from build123d import *

# Parameters (mm, degrees)
M4_TAPPED_HOLE1_D     = 3.3
M4_TAPPED_HOLE1_DEPTH = 9.8
M4_TAPPED_HOLE1_TIP   = 0.991420021
CHAMFER1_SIZE         = 1


with BuildPart() as part:
    # Sketch1 → Revolve1 (revolve)
    with BuildSketch(Plane.XY, mode=Mode.PRIVATE) as revolve1_sk:
        Polygon((25, 0), (46.5, 0), (46.5, 4), (42.5, 4), (42.5, 14.5), (25, 14.5), align=None)
    revolve(revolve1_sk.sketch.rotate(Axis((0, 0, 0), (0, 1, 0)), 90), axis=Axis((0, 0, 0), (0, 1, 0)))

    # M4 Tapped Hole1
    with Locations(Plane(origin=(0, 0, 0), x_dir=(-1, 0, 0), z_dir=(0, -1, 0))):
        with Locations((0, -36.5), (-31.609927238, -18.25), (-31.609927238, 18.25), (0, 36.5), (31.609927238, 18.25), (31.609927238, -18.25)):
            Hole(M4_TAPPED_HOLE1_D / 2, depth=M4_TAPPED_HOLE1_DEPTH)
            with Locations((0, 0, -(M4_TAPPED_HOLE1_DEPTH + M4_TAPPED_HOLE1_TIP / 2))):  # 118° drill point
                Cone(0, M4_TAPPED_HOLE1_D / 2, M4_TAPPED_HOLE1_TIP, mode=Mode.SUBTRACT)

    # Chamfer1
    chamfer1_edges = [part.edges().sort_by_distance(p)[0] for p in [
        (0, 0, 25),
        (0, 14.5, 25),
        (0, 14.5, 42.5),
    ]]
    chamfer(chamfer1_edges, length=CHAMFER1_SIZE)


solid = part.part
Source: CAD feature listing. Evaluate the final solid. Frame: model axes, mm. A direction names the side the tool comes from. Give positions to 0.01 mm unless a question says otherwise; leave off trailing zeros. Order: outer loops, then holes, each group sorted by start corner. A loop starts at its lowest first (then second) coordinate and runs counter-clockwise, first axis right, second up. Notation, with made-up numbers: (33, 40) -> (47, 40) arc R25 cw to (47, 73) -> close; hole circle Ø7 at (72.5, -32.75). An arc over 180 degrees is marked (long way). Write item = value, one per line.
Item 1: Section query A-A (z = 0). Output: boundary loops of the cut face in (x, y), then the cut area to 4 significant figures.
Check result:
outline = (-46.5, 0) -> (-26, 0) -> (-25, 1) -> (-25, 13.5) -> (-26, 14.5) -> (-41.5, 14.5) -> (-42.5, 13.5) -> (-42.5, 4) -> (-46.5, 4) -> close; (25, 1) -> (26, 0) -> (46.5, 0) -> (46.5, 4) -> (42.5, 4) -> (42.5, 13.5) -> (41.5, 14.5) -> (26, 14.5) -> (25, 13.5) -> close
area = 536.5 mm²
Item 2: Mould query, pull axis X, two halves, no side actions, for faces 1 (the face through (-33.26, 4.97, -18.32)), 2 (the face through (33.184, 4.969, -18.746)), 3 (the face through (18, 14.5, 19)), 4 (the face through (-12.766, 8.817, -40.537)). Classes: +X half, -X half, draft (parallel to the pull), parting line (faces both ways), or undercut.
Check result:
face_1 = undercut
face_2 = undercut
face_3 = draft
face_4 = parting line
Item 3: Ray query, probe 1 along X at (y, z) = (7.5, -18.25); probe 2 along X at (y, z) = (6.5, -17.5); probe 3 along Z at (x, y) = (33, 4.75). Return the intervals inside material, ascending.
Check result:
probe_1 = -38.38 to -33.26, -29.96 to -17.09, 17.09 to 29.96, 33.26 to 38.38
probe_2 = -38.73 to -33.08, -30.14 to -17.85, 17.85 to 30.14, 33.08 to 38.73
probe_3 = -26.78 to -19.14, -17.36 to 17.36, 19.14 to 26.78
Item 4: Contact query for flat-ended pins moving along their axis: pin 1 (2 mm diameter, centred on x = 0, z = -36.5, fed in from -Y); pin 2 (3 mm diameter, centred on x = -10.5, y = 2, fed in from +Z); pin 3 (3 mm diameter, centred on x = -31.61, z = 18.25, fed in from -Y). Output: stop coordinate, or through.
Check result:
pin_1 = 10.19
pin_2 = 45.62
pin_3 = 9.89
Item 5: Set-up query: faces 5 (the face through (-33.26, 4.97, 18.18)), 6 (the face through (20, 0, 20)), 7 (the face through (38, 4, -20)). Return all of +Z, -Z, +X, -X, +Y, -Y with unobstructed straight access to the full face (end or side cutting, diameter ignored); none if empty.
Check result:
face_5 = -Y
face_6 = +Z, -Z, +X, -X, -Y
face_7 = +Y
Item 6: Section query B-B (y = 5.25). Output: boundary loops of the cut face in (x, z), then the cut area to 3 significant figures.
Check result:
outline = circle Ø85 at (0, 0); hole circle Ø3.3 at (-31.61, -18.25); hole circle Ø3.3 at (-31.61, 18.25); hole circle Ø50 at (0, 0); hole circle Ø3.3 at (0, -36.5); hole circle Ø3.3 at (0, 36.5); hole circle Ø3.3 at (31.61, -18.25); hole circle Ø3.3 at (31.61, 18.25)
area = 3,660 mm²
